Here's how the part is built. I have some questions about the finished solid (model axes, mm). A direction names the side the tool comes from. Round coordinates to 2 decimals unless told otherwise and drop trailing zeros. Return JSON: item names as keys, results as strings. Group by question number.
```python
from build123d import *

# Parameters (mm, degrees)
EXTRUDE_642_DEPTH   = 1648
SKETCH_2_W          = 64
SKETCH_2_H          = 64
EXTRUDE_1_DEPTH     = 85
SKETCH_4_W          = 54
SKETCH_4_H          = 12
EXTRUDE_2_DEPTH     = 10
CUT_EXTRUDE_1_DEPTH = 10
SKETCH_6_W          = 64
SKETCH_6_H          = 69
EXTRUDE_3_DEPTH     = 15
SKETCH_7_W          = 48
SKETCH_7_H          = 88
EXTRUDE_4_DEPTH     = 88
SKETCH_8_R          = 36.5
CUT_EXTRUDE_2_DEPTH = 3
SKETCH_9_R          = 8
EXTRUDE_5_DEPTH     = 19


with BuildPart() as part:
    # 草图1 → Extrude 642 (new body)
    with BuildSketch(Plane.XY):
        Polygon((9.931917842, 6.925864063), (9.931917842, 41.925864063), (12.931917842, 41.925864063), (12.931917842, 40.425864063), (16.931917842, 40.425864063), (16.931917842, 48.425864063), (12.931917842, 48.425864063), (12.931917842, 46.925864063), (9.931917842, 46.925864063), (9.931917842, 56.425864063), (73.931917842, 56.425864063), (73.931917842, 46.925864063), (70.931917842, 46.925864063), (70.931917842, 48.425864063), (66.931917842, 48.425864063), (66.931917842, 40.425864063), (70.931917842, 40.425864063), (70.931917842, 41.925864063), (73.931917842, 41.925864063), (73.931917842, 6.925864063), (70.931917842, 6.925864063), (70.931917842, 8.425864063), (66.931917842, 8.425864063), (66.931917842, 0.425864063), (70.931917842, 0.425864063), (70.931917842, 1.925864063), (73.931917842, 1.925864063), (73.931917842, -7.574135937), (9.931917842, -7.574135937), (9.931917842, 1.925864063), (12.931917842, 1.925864063), (12.931917842, 0.425864063), (16.931917842, 0.425864063), (16.931917842, 8.425864063), (12.931917842, 8.425864063), (12.931917842, 6.925864063), align=None)
    extrude(amount=-EXTRUDE_642_DEPTH)

    # 草图2 → 凸台-拉伸1 (add)
    with BuildSketch(Plane.XY):
        with Locations((41.931917842, 24.425864063)):
            Rectangle(SKETCH_2_W, SKETCH_2_H)
    extrude(amount=EXTRUDE_1_DEPTH)

    # 草图4 → 凸台-拉伸2 (add)
    with BuildSketch(Plane(origin=(0, 56.425864063, 0), x_dir=(-1, 0, 0), z_dir=(0, 1, 0))):
        with Locations((-41.931917842, 6)):
            Rectangle(SKETCH_4_W, SKETCH_4_H)
    extrude(amount=EXTRUDE_2_DEPTH)

    # 草图5 → 切除-拉伸1 (cut)
    with BuildSketch(Plane(origin=(73.931917842, 0, 0), x_dir=(0, 0, -1), z_dir=(1, 0, 0))):
        with BuildLine():
            Line((0, 48.925864063), (-6, 48.925864063))
            ThreePointArc((-6, 48.925864063), (-8.828427125, 47.754291188), (-10, 44.925864063))
            Line((-10, 44.925864063), (-10, 43.925864063))
            ThreePointArc((-10, 43.925864063), (-8.828427125, 41.097436938), (-6, 39.925864063))
            Line((-6, 39.925864063), (0, 39.925864063))
            Line((0, 39.925864063), (0, 48.925864063))
        make_face()
        with BuildLine():
            Line((0, 8.925864063), (-6, 8.925864063))
            ThreePointArc((-6, 8.925864063), (-8.828427125, 7.754291188), (-10, 4.925864063))
            Line((-10, 4.925864063), (-10, 3.925864063))
            ThreePointArc((-10, 3.925864063), (-8.828427125, 1.097436938), (-6, -0.074135937))
            Line((-6, -0.074135937), (0, -0.074135937))
            Line((0, -0.074135937), (0, 8.925864063))
        make_face()
    cut_extrude_1 = extrude(amount=-CUT_EXTRUDE_1_DEPTH, mode=Mode.SUBTRACT)

    # 镜向1: 切除-拉伸1 across plane
    add(cut_extrude_1.mirror(Plane.ZY.offset(-41.931917842)), mode=Mode.SUBTRACT)

    # 草图6 → 凸台-拉伸3 (add)
    with BuildSketch(Plane(origin=(0, 0, -1648), x_dir=(-1, 0, 0), z_dir=(0, 0, -1))):
        with Locations((-41.931917842, 26.925864063)):
            Rectangle(SKETCH_6_W, SKETCH_6_H)
    extrude(amount=EXTRUDE_3_DEPTH)

    # 草图7 → 凸台-拉伸4 (add)
    with BuildSketch(Plane(origin=(0, 0, -1663), x_dir=(-1, 0, 0), z_dir=(0, 0, -1))):
        with Locations((-41.931917842, 24.425864063)):
            Rectangle(SKETCH_7_W, SKETCH_7_H)
    extrude(amount=EXTRUDE_4_DEPTH)

    # 草图8 → 切除-拉伸2 (cut)
    with BuildSketch(Plane.ZY.offset(-17.931917842)):
        with Locations((-1707, 24.425864063)):
            Circle(SKETCH_8_R)
    extrude(amount=-CUT_EXTRUDE_2_DEPTH, mode=Mode.SUBTRACT)

    # 草图9 → 凸台-拉伸5 (add)
    with BuildSketch(Plane.ZY.offset(-20.931917842)):
        with Locations((-1707, 24.425864063)):
            Circle(SKETCH_9_R)
    extrude(amount=EXTRUDE_5_DEPTH)


solid = part.part
```
Q1. Please list where these lines run through material, in increasing order: line 1 (Y direction, x = 19.2, z = -1707); line 2 (X direction, y = 7.5, z = -209.5); line 3 (Z direction, x = 16.5, y = 23).
Q2. Will these pins go through, and if not, where does the flat tip stop? pin 1 Ø1.5 at (x, z) = (13.5, -363) entering from -Y; pin 2 Ø2.5 at (x, z) = (72.5, -1045) entering from +Y; pin 3 Ø6 at (x, z) = (44.5, 8) entering from +Y.
Q3. For faces 1 (the flat face through (42, -19.574, -1706)), 2 (the flat face through (42, -7.574, -777)), 3 (the flat face through (20.932, 25, -1716)), 4 (the flat face through (65.932, 24, -1706)), which set-ups out of +Z, -Z, +X, -X, +Y, -Y let a thin tool reach every point of the face, with its end or its side?
Q4. If we mould it in two halves opening along Z, with no side actions, what happens to faces 5 (the flat face through (41, 56.426, -794)), 6 (the flat face through (42, 25, -1751)), 7 (the cylindrical face through (19.411, 26.031, -1743.465)), 8 (the flat face through (9.932, 26, -777))? For each: +Z half, -Z half, draft (parallel to the pull), parting line (faces both ways), or undercut.
Output values:
{
 "1": {"line 1": "y = -19.57 to -12.07, 16.43 to 32.43, 60.93 to 68.43", "line 2": "x = 9.93 to 12.93, 16.93 to 66.93, 70.93 to 73.93", "line 3": "z = -1714.87 to -1699.13, -1663 to 85"},
 "2": {"pin 1": "stops at y = -7.57", "pin 2": "stops at y = 56.43", "pin 3": "stops at y = 66.43"},
 "3": {"face 1": "+Z, -Z, +X, -X, -Y", "face 2": "+Z, +X, -X, -Y", "face 3": "-X", "face 4": "-Z, +X, +Y, -Y"},
 "4": {"face 5": "undercut", "face 6": "-Z half", "face 7": "undercut", "face 8": "draft"}
}
